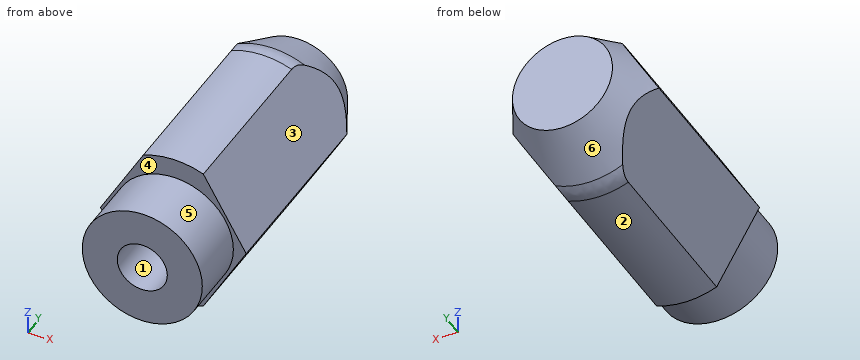
```python
from build123d import *

# Parameters (mm, degrees)
M3_TAPPED_HOLE1_D     = 2.5
M3_TAPPED_HOLE1_DEPTH = 10
M3_TAPPED_HOLE1_TIP   = 0.751075774
CUT_EXTRUDE1_DEPTH    = 17.031219542
FILLET1_R             = 2


with BuildPart() as part:
    # Sketch1 → Revolve1 (revolve)
    with BuildSketch(Plane.XY):
        Polygon((0, 0), (0, 15), (2.5, 15), (4, 12), (4, 3), (3, 3), (3, 0), align=None)
    revolve(axis=Axis((0, 0, 0), (0, 1, 0)))

    # M3 Tapped Hole1
    with Locations(Plane(origin=(0, 0, 0), x_dir=(-1, 0, 0), z_dir=(0, -1, 0))):
        with Locations((0, 0)):
            Hole(M3_TAPPED_HOLE1_D / 2, depth=M3_TAPPED_HOLE1_DEPTH)
            with Locations((0, 0, -(M3_TAPPED_HOLE1_DEPTH + M3_TAPPED_HOLE1_TIP / 2))):  # 118° drill point
                Cone(0, M3_TAPPED_HOLE1_D / 2, M3_TAPPED_HOLE1_TIP, mode=Mode.SUBTRACT)

    # Sketch4 → Cut-Extrude1 (cut, through all)
    with BuildSketch(Plane(origin=(0, 15, 0), x_dir=(1, 0, 0), z_dir=(0, 1, 0))):
        with BuildLine():
            Line((-1.5, 3.708099244), (-3.640872096, 0))
            Line((-3.640872096, 0), (-1.5, -3.708099244))
            ThreePointArc((-1.5, -3.708099244), (-4, 0), (-1.5, 3.708099244))
        make_face()
        with BuildLine():
            Line((1.5, 3.708099244), (3.640872096, 0))
            Line((3.640872096, 0), (1.5, -3.708099244))
            ThreePointArc((1.5, -3.708099244), (4, 0), (1.5, 3.708099244))
        make_face()
    extrude(amount=-CUT_EXTRUDE1_DEPTH, mode=Mode.SUBTRACT)

    # Fillet1
    fillet1_edges = [part.edges().sort_by_distance(p)[0] for p in [
        (0, 12, -4),
        (0, 12, 4),
    ]]
    fillet(fillet1_edges, radius=FILLET1_R)


solid = part.part
```
Design review of the part built by this model. Coordinates are the model's own, in mm. Face numbers are marked on the shaded views. A direction names the side the tool comes from. Coordinates: 2 decimals unless noted, no trailing zeros. Order: outer loops, then holes, each group sorted by start corner. A loop starts at its lowest first (then second) coordinate and runs counter-clockwise, first axis right, second up. Notation, with made-up numbers: (73, 64) - (84, 64) arc R6 cw to (84, 69) - close; hole circle Ø8 at (-23, 73). An arc over 180 degrees is marked (long way). Answer in a Markdown table with one row per item.
(1) Clearance check with a flat-ended pin moving along its axis: pin 1 (3 mm diameter, centred on x = 0, z = 0, fed in from -Y). State where the tip first meets the part, or that it passes through.
Checked values:
| item | result |
|---|---|
| pin 1 | y = 0 |
(2) Wall thickness on line 1 along Z through (x, y) = (0, 2); line 2 along Z through (x, y) = (0, 5.5); line 3 along Y through (x, z) = (-2.5, -0.5): over which ranges is each line inside the solid? List them lowest first. Write a range as from..to.
Checked values:
| item | result |
|---|---|
| line 1 | -3..-1.25, 1.25..3 |
| line 2 | -4..-1.25, 1.25..4 |
| line 3 | 0..14.9 |
(3) For the marked faces 5 and 6, list the 3-axis set-ups (+Z, -Z, +X, -X, +Y, -Y) from which the entire face can be reached by the end or side of a thin tool; tool diameter is ignored.
Checked values:
| item | result |
|---|---|
| face 5 | -Y |
| face 6 | +Y |
(4) The part is to be moulded in two halves that separate along Z. For the marked faces 1, 2, 3 and 4, say which applies: released by +Z, released by -Z, zero draft, split by the parting line, or undercut.
Checked values:
| item | result |
|---|---|
| face 1 | undercut |
| face 2 | released by -Z |
| face 3 | released by +Z |
| face 4 | zero draft |
(5) Consider section A-A on y = 7.25. State the section outline as (x, z) points, plus the area to 3 significant figures.
Checked values:
| item | result |
|---|---|
| outline | (-3.64, 0) - (-1.5, -3.71) arc R4 ccw to (1.5, -3.71) - (3.64, 0) - (1.5, 3.71) arc R4 ccw to (-1.5, 3.71) - close; hole circle Ø2.5 at (0, 0) |
| area | 34.4 mm^2 |
(6) Consider section B-B on y = 2.5. State the section outline as (x, z) points.
Checked values:
| item | result |
|---|---|
| outline | circle Ø6 at (0, 0); hole circle Ø2.5 at (0, 0) |
